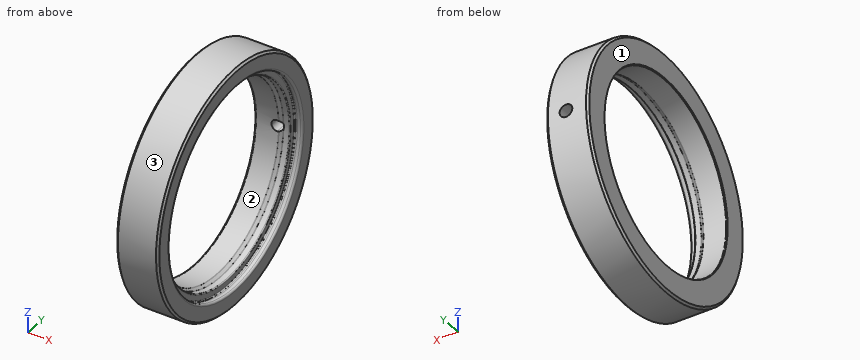
from build123d import *
from build123d.topology import SkipClean

# Parameters (mm, degrees)
CHAMFER2_SIZE                      = 0.762
CHAMFER2_SIZE2                     = 0.439940905
CHAMFER3_SIZE                      = 1.524
F_1_8_NPT_TAPPED_HOLE1_D           = 8.636
F_1_8_NPT_TAPPED_HOLE1_DEPTH       = 19.431
F_1_8_NPT_TAPPED_HOLE1_CBORE_D     = 9.6527874
F_1_8_NPT_TAPPED_HOLE1_CBORE_DEPTH = 9.652
F_1_8_NPT_TAPPED_HOLE1_TIP         = 2.594516153
SKETCH4_R                          = 4.318
CUT_EXTRUDE1_DEPTH                 = 82.423


with BuildPart() as part:
    # Sketch1 → Revolve1 (revolve)
    with BuildSketch(Plane.XY, mode=Mode.PRIVATE) as revolve1_sk:
        with BuildLine():
            Line((0, 92.075), (32, 92.075))
            Line((32, 92.075), (32, 80.044))
            ThreePointArc((32, 80.044), (31.553630735, 78.966369265), (30.476, 78.52))
            Line((30.476, 78.52), (28.075925561, 78.52))
            Line((28.075925561, 78.52), (26.559220112, 78.9264))
            ThreePointArc((26.559220112, 78.9264), (25.898123791, 78.794899766), (25.6, 78.19036452))
            Line((25.6, 78.19036452), (25.6, 74.422))
            ThreePointArc((25.6, 74.422), (25.376815367, 73.883184633), (24.838, 73.66))
            Line((24.838, 73.66), (20.785834534, 73.66))
            ThreePointArc((20.785834534, 73.66), (20.588614422, 73.63403548), (20.404834534, 73.557911358))
            Line((20.404834534, 73.557911358), (18.206822715, 72.288888642))
            ThreePointArc((18.206822715, 72.288888642), (18.023042828, 72.21276452), (17.825822715, 72.1868))
            Line((17.825822715, 72.1868), (0, 72.1868))
            Line((0, 72.1868), (0, 92.075))
        make_face()
    revolve(revolve1_sk.sketch.rotate(Axis((-48.080119454, 0, 0), (1, 0, 0)), 90), axis=Axis((-48.080119454, 0, 0), (1, 0, 0)))

    # Chamfer2
    chamfer2_edges = [part.edges().sort_by_distance(p)[0] for p in [
        (0, 0, -72.1868),
    ]]
    chamfer2_side = [part.faces().sort_by_distance(p)[0] for p in [
        (8.912911358, 0, -72.1868),
    ]]
    chamfer(chamfer2_edges, length=CHAMFER2_SIZE, length2=CHAMFER2_SIZE2, reference=chamfer2_side[0])

    # Chamfer3
    chamfer3_edges = [part.edges().sort_by_distance(p)[0] for p in [
        (32, 0, -92.075),
        (0, 0, -92.075),
    ]]
    chamfer(chamfer3_edges, length=CHAMFER3_SIZE)

    # 1/8 NPT Tapped Hole1
    with Locations(Plane(origin=(16.76, 92.075, 0), x_dir=(0, 0, 1), z_dir=(0, 1, 0))):
        with Locations((0, 0)):
            CounterBoreHole(F_1_8_NPT_TAPPED_HOLE1_D / 2, F_1_8_NPT_TAPPED_HOLE1_CBORE_D / 2, F_1_8_NPT_TAPPED_HOLE1_CBORE_DEPTH, depth=F_1_8_NPT_TAPPED_HOLE1_DEPTH)
            with Locations((0, 0, -(F_1_8_NPT_TAPPED_HOLE1_DEPTH + F_1_8_NPT_TAPPED_HOLE1_TIP / 2))):  # 118° drill point
                Cone(0, F_1_8_NPT_TAPPED_HOLE1_D / 2, F_1_8_NPT_TAPPED_HOLE1_TIP, mode=Mode.SUBTRACT)

    # Sketch4 → Cut-Extrude1 (cut)
    with SkipClean():  # the faces are left unmerged after this step: merging them gives an invalid solid
        with BuildSketch(Plane(origin=(0, 0, 0), x_dir=(1, 0, 0), z_dir=(0, 1, 0))):
            with Locations(Location((16.76, 0, 0), (0, 0, 270))):
                Circle(SKETCH4_R)
        extrude(amount=CUT_EXTRUDE1_DEPTH, mode=Mode.SUBTRACT)


solid = part.part
Can you work these out from the model? Positions are in its coordinate system, mm. Face numbers are marked on the shaded views. Give positions to 0.01 mm unless a question says otherwise; leave off trailing zeros. One line per item, written item: value.
1) Please list where these lines run through material, in increasing order: line 1 (Y direction, x = 10, z = 0) (3 decimals); line 2 (Y direction, x = 20, z = 13); line 3 (Z direction, x = 6, y = -51).
Geometry check:
line 1: y = -92.075 to -72.187, 72.187 to 92.075
line 2: y = -91.15 to -72.16, 72.16 to 91.15
line 3: z = -76.66 to -51.09, 51.09 to 76.66
2) Thinking about a two-plate mould opening in Z: for the marked faces 1, 2 and 3, which applies, +Z half, -Z half, draft (parallel to the pull), parting line (faces both ways), or undercut?
Geometry check:
face 1: draft
face 2: undercut
face 3: parting line
3) I'm going to push flat-ended pins straight in: pin 1 (1 mm diameter, centred on x = 27, z = -16, fed in from +Y); pin 2 (10 mm diameter, centred on x = 27, y = -32.5, fed in from +Z); pin 3 (8 mm diameter, centred on x = 6.5, z = 49, fed in from +Y). Where does each tip first touch, or does it pass through?
Geometry check:
pin 1: stops at y = 90.76
pin 2: stops at z = 87.87
pin 3: stops at y = 80.33
